from build123d import *

# Parameters (mm, degrees)
HOUSING_BODY_60_DEPTH        = 60
LIFTING_START                = -10
LIFTING_LUG_SKETCH_R         = 5
LIFTING_LUG_DEPTH            = 10
MOUNTING_FLANGES_SKETCH_W    = 20
MOUNTING_FLANGES_SKETCH_H    = 48
MOUNTING_FLANGES_SKETCH_R    = 5
MOUNTING_FLANGES_14_DEPTH    = 14
FLANGE_CORNER_FILLET_R10_A_R = 10
FLANGE_CORNER_FILLET_R10_B_R = 10
FLANGE_CORNER_FILLET_R10_C_R = 10
FLANGE_CORNER_FILLET_R10_D_R = 10
TOP_RECESS_4_DEEP_DEPTH      = 4
RECESS_HOLE_SKETCH_R         = 5
RECESS_HOLE_DEPTH            = 145.211650056


with BuildPart() as part:
    # Body Profile Sketch → Housing Body 60 (new body)
    with BuildSketch(Plane.XY):
        with BuildLine():
            Line((0, 0), (0, 70))
            ThreePointArc((0, 70), (33, 103), (66, 70))
            Line((66, 70), (66, 0))
            Line((66, 0), (46, 0))
            Line((46, 0), (46, 70))
            ThreePointArc((46, 70), (33, 83), (20, 70))
            Line((20, 70), (20, 0))
            Line((20, 0), (0, 0))
        make_face()
    extrude(amount=-HOUSING_BODY_60_DEPTH)

    # Lifting Lug Sketch → Lifting Lug (add)
    with BuildSketch(Plane(origin=(0, 0, -60), x_dir=(-1, 0, 0), z_dir=(0, 0, -1)).offset(LIFTING_START)):
        with BuildLine():
            Line((-43, 101.448370387), (-43, 111.448370387))
            ThreePointArc((-43, 111.448370387), (-33, 121.448370387), (-23, 111.448370387))
            Line((-23, 111.448370387), (-23, 101.448370387))
            ThreePointArc((-23, 101.448370387), (-33, 103), (-43, 101.448370387))
        make_face()
        with Locations((-33, 111.448370387)):
            Circle(LIFTING_LUG_SKETCH_R, mode=Mode.SUBTRACT)
    extrude(amount=LIFTING_LUG_DEPTH)

    # Mounting Flanges Sketch → Mounting Flanges 14 (add)
    # profile 1 of 2: a face of its own
    with BuildSketch(Plane(origin=(0, 70, 0), x_dir=(1, 0, 0), z_dir=(0, 1, 0))):
        with Locations((76, 30)):
            Rectangle(MOUNTING_FLANGES_SKETCH_W, MOUNTING_FLANGES_SKETCH_H)
        with Locations(Location((76, 20, 0), (0, 0, 270))):
            Circle(MOUNTING_FLANGES_SKETCH_R, mode=Mode.SUBTRACT)
        with Locations(Location((76, 40, 0), (0, 0, 270))):
            Circle(MOUNTING_FLANGES_SKETCH_R, mode=Mode.SUBTRACT)
    # profile 2 of 2: a face of its own
    with BuildSketch(Plane(origin=(0, 70, 0), x_dir=(1, 0, 0), z_dir=(0, 1, 0))):
        with Locations((-10, 30)):
            Rectangle(MOUNTING_FLANGES_SKETCH_W, MOUNTING_FLANGES_SKETCH_H)
        with Locations(Location((-10, 40, 0), (0, 0, 90))):
            Circle(MOUNTING_FLANGES_SKETCH_R, mode=Mode.SUBTRACT)
        with Locations(Location((-10, 20, 0), (0, 0, 90))):
            Circle(MOUNTING_FLANGES_SKETCH_R, mode=Mode.SUBTRACT)
    extrude(amount=-MOUNTING_FLANGES_14_DEPTH)

    # Flange Corner Fillet R10 A
    flange_corner_fillet_r10_a_edges = [part.edges().sort_by_distance(p)[0] for p in [
        (86, 63, -54),
    ]]
    fillet(flange_corner_fillet_r10_a_edges, radius=FLANGE_CORNER_FILLET_R10_A_R)

    # Flange Corner Fillet R10 B
    flange_corner_fillet_r10_b_edges = [part.edges().sort_by_distance(p)[0] for p in [
        (86, 63, -6),
    ]]
    fillet(flange_corner_fillet_r10_b_edges, radius=FLANGE_CORNER_FILLET_R10_B_R)

    # Flange Corner Fillet R10 C
    flange_corner_fillet_r10_c_edges = [part.edges().sort_by_distance(p)[0] for p in [
        (-20, 63, -54),
    ]]
    fillet(flange_corner_fillet_r10_c_edges, radius=FLANGE_CORNER_FILLET_R10_C_R)

    # Flange Corner Fillet R10 D
    flange_corner_fillet_r10_d_edges = [part.edges().sort_by_distance(p)[0] for p in [
        (-20, 63, -6),
    ]]
    fillet(flange_corner_fillet_r10_d_edges, radius=FLANGE_CORNER_FILLET_R10_D_R)

    # Top Recess Sketch → Top Recess 4 Deep (cut)
    with BuildSketch(Plane(origin=(0, 103, 0), x_dir=(1, 0, 0), z_dir=(0, 1, 0))):
        with BuildLine():
            Line((21.724814581, 43), (21.724814581, 17))
            ThreePointArc((21.724814581, 17), (33, 18.894718879), (44.244993393, 16.828347794))
            Line((44.244993393, 16.828347794), (44.244993393, 42.828347794))
            ThreePointArc((44.244993393, 42.828347794), (33, 44.894718879), (21.724814581, 43))
        make_face()
    extrude(amount=-TOP_RECESS_4_DEEP_DEPTH, mode=Mode.SUBTRACT)

    # Recess Hole Sketch → Recess Hole (cut, through all)
    with BuildSketch(Plane(origin=(0, 99, 0), x_dir=(1, 0, 0), z_dir=(0, 1, 0))):
        with Locations(Location((33.108870808, 31.892430073, 0), (0, 0, 180))):
            Circle(RECESS_HOLE_SKETCH_R)
    extrude(amount=-RECESS_HOLE_DEPTH, mode=Mode.SUBTRACT)


solid = part.part
The listing builds one solid part. Answer for the finished solid, in the listing's coordinates (mm). A direction names the side the tool comes from. Coordinates: 2 decimals unless noted, no trailing zeros. Loops run counter-clockwise (first coordinate to the right, second up) from the corner with the lowest first, then second, coordinate; pieces in that order, holes last. Notation, with made-up numbers: (77.5, 18) -> (85.5, 18) arc R10 cw to (85.5, 22) -> close; hole circle Ø4 at (66.25, 39.5). An arc over 180 degrees is marked (long way). Answer in a Markdown table with one row per item. Add a question column.
1. For faces 4 (the flat face through (23, 107, -55)), 5 (the flat face through (20, 35, -30)), 6 (the flat face through (-10, 56, -30)), 7 (the flat face through (-5, 63, -54)), determine the directions among +Z, -Z, +X, -X, +Y, -Y from which every point of the face is accessible in a straight line to the end or side of a thin tool.
2. The part is cut by section C-C, the plane y = 29. Write down the section's boundary in (x, z), then the cut area to 3 significant figures.
3. Consider line 1 (X direction, y = 66, z = -20); line 2 (X direction, y = 10.5, z = -20); line 3 (X direction, y = 96.5, z = -31.5). Determine where each line is inside the solid, lowest interval first. Write a range as [from, to].
4. Determine the mould class of faces 1 (the cylindrical face through (-16.99, 62.9, -51.15)), 2 (the cylindrical face through (-14.957, 63.098, -19.349)), 3 (the flat face through (66, 28, -30)) for opening direction Z: +Z half, -Z half, draft (parallel to the pull), parting line (faces both ways), or undercut.
5. The part is cut by section B-B, the plane z = -56. Write down the section's boundary in (x, y).
6. The part is cut by section D-D, the plane x = 33. Write down the section's boundary in (y, z), then the cut area to 3 significant figures.
7. Flat-ended cylindrical pins translate along their axes: P1, Ø25, axis at x = 35.5, z = -24.5, coming from the +Y side; P2, Ø6, axis at x = -9.5, z = -41.5, coming from the +Y side; P3, Ø5, axis at y = 99, z = -36.5, coming from the -X side; P4, Ø8, axis at x = 73, y = 61, coming from the +Z side. Find the tip coordinate at first contact, or state that the pin passes through.
8. The part is cut by section A-A, the plane z = -40. Write down the section's boundary in (x, y) (3 decimals).
Answer below:
| question | item | result |
|---|---|---|
| 1 | face 4 | +Z, -Z, -X, +Y |
| 1 | face 5 | +Z, -Z, -Y |
| 1 | face 6 | +Z, -Z, -X, -Y |
| 1 | face 7 | -Z, -X, +Y, -Y |
| 2 | outline | (0, -60) -> (20, -60) -> (20, 0) -> (0, 0) -> close; (46, -60) -> (66, -60) -> (66, 0) -> (46, 0) -> close |
| 2 | area | 2,400 mm2 |
| 3 | line 1 | [-20, -15], [-5, 20], [46, 71], [81, 86] |
| 3 | line 2 | [0, 20], [46, 66] |
| 3 | line 3 | [13.33, 28.12], [38.09, 52.67] |
| 4 | face 1 | -Z half |
| 4 | face 2 | undercut |
| 4 | face 3 | draft |
| 5 | outline | (0, 0) -> (20, 0) -> (20, 70) arc R13 cw to (46, 70) -> (46, 0) -> (66, 0) -> (66, 70) arc R33 ccw to (43, 101.45) -> (43, 111.45) arc R10 ccw to (23, 111.45) -> (23, 101.45) arc R33 ccw to (0, 70) -> close; hole circle Ø10 at (33, 111.45) |
| 6 | outline | (83, -60) -> (106.45, -60) -> (106.45, -50) -> (103, -50) -> (103, -44.89) -> (99, -44.89) -> (99, -36.89) -> (83, -36.89) -> close; (83, -26.89) -> (99, -26.89) -> (99, -18.89) -> (103, -18.89) -> (103, 0) -> (83, 0) -> close; (116.45, -60) -> (121.45, -60) -> (121.45, -50) -> (116.45, -50) -> close |
| 6 | area | 1,020 mm2 |
| 7 | P1 | y = 103 |
| 7 | P2 | through |
| 7 | P3 | x = 13.33 |
| 7 | P4 | z = -6 |
| 8 | outline | (-20, 56) -> (-15, 56) -> (-15, 70) -> (-20, 70) -> close; (-5, 56) -> (0, 56) -> (0, 0) -> (20, 0) -> (20, 70) arc R13 cw to (46, 70) -> (46, 0) -> (66, 0) -> (66, 56) -> (71, 56) -> (71, 70) -> (66, 70) arc R33 ccw to (44.245, 101.025) -> (44.245, 99) -> (21.725, 99) -> (21.725, 101.014) arc R33 ccw to (0, 70) -> (-5, 70) -> close; (81, 56) -> (86, 56) -> (86, 70) -> (81, 70) -> close |
